Could you check a few things on this model? Use its own coordinates, in mm. A direction names the side the tool comes from. Give positions to 0.01 mm unless a question says otherwise; leave off trailing zeros. Order: outer loops, then holes, each group sorted by start corner. A loop starts at its lowest first (then second) coordinate and runs counter-clockwise, first axis right, second up. Notation, with made-up numbers: M 86.5,64.25 L 124.5,64.25 A27 cw 124.5,102.25 Z; hole C 52,46 d11. An arc over 180 degrees is marked long. Return JSON: item names as keys, results as strings. Group by question number.
```python
from build123d import *

# Parameters (mm, degrees)
CUT_EXTRUDE1_REACH = 152
SKETCH2_W          = 12
SKETCH2_H          = 6.6


with BuildPart() as part:
    # Sketch1 → Revolve1 (revolve)
    with BuildSketch(Plane.XY, mode=Mode.PRIVATE) as revolve1_sk:
        Polygon((-25, 21), (25, 21), (25, 30), (5, 30), (5, 90), (25, 90), (25, 100), (-25, 100), (-25, 90), (-5, 90), (-5, 30), (-25, 30), align=None)
    revolve(revolve1_sk.sketch.rotate(Axis((0, 0, 0), (1, 0, 0)), 90), axis=Axis((0, 0, 0), (1, 0, 0)))

    # Sketch2 → Cut-Extrude1 (cut, up to next)
    with BuildSketch(Plane(origin=(25, 0, 0), x_dir=(0, 0, -1), z_dir=(1, 0, 0)), mode=Mode.PRIVATE) as cut_extrude1_sk1:
        with Locations((0, 21)):
            Rectangle(SKETCH2_W, SKETCH2_H)
    cut_extrude1_tool1 = extrude(cut_extrude1_sk1.sketch, amount=-CUT_EXTRUDE1_REACH, mode=Mode.PRIVATE) & part.part
    add(cut_extrude1_tool1.solids().sort_by_distance((25, 21, 0))[0], mode=Mode.SUBTRACT)


solid = part.part
```
1. For pin 1 (25 mm diameter, centred on y = 0, z = 0, fed in from -X); pin 2 (3 mm diameter, centred on x = -11.5, z = -21.5, fed in from -Y); pin 3 (12 mm diameter, centred on x = -18.5, y = 41.5, fed in from -Z); pin 4 (1.5 mm diameter, centred on x = 19.5, z = -79.5, fed in from -Y), each with a flat end and sliding along its axis, tell me the tip position at first contact or that it passes through.
2. Imagine slicing it at A-A, the plane y = 0. Please give me the cut outline in (x, z), plus the area to 3 significant figures.
3. Imagine slicing it at D-D, the plane z = 77. Please give me the cut outline in (x, y), plus the area to 3 significant figures.
4. Imagine slicing it at B-B, the plane x = 15. Please give me the cut outline in (y, z).
5. Which directions (+Z, -Z, +X, -X, +Y, -Y) give clear straight access to the entire face, cutting with the end or side of a thin tool? Please do faces 4 (the cylindrical face through (14.86, -25.296, 16.128)), 5 (the flat face through (25, -20.4, -6.2)), 6 (the flat face through (0, 24.3, 0)), 7 (the flat face through (-5, 39, -1)).
6. I need wall thicknesses on L1, parallel to Y at x = -22, z = -0.5; L2, parallel to Z at x = 18, y = -3; L3, parallel to Z at x = -16, y = -9. Which ranges of each line are inside material? Lowest first, please. Write a range as from..to.
7. Imagine slicing it at C-C, the plane z = 0. Please give me the cut outline in (x, y).
8. If we mould it in two halves opening along Z, with no side actions, what happens to faces 1 (the cylindrical face through (0.35, -20.983, 0.838)), 2 (the cylindrical face through (-0.35, -30.04, 95.38)), 3 (the flat face through (-25, -38, -82))? For each: pulls with the +Z half, pulls with the -Z half, needs draft (parallel to the pull), parting line crosses it, or undercut.
Values:
{
 "1": {"pin 1": "passes through", "pin 2": "stops at y = -97.98", "pin 3": "stops at z = -93.49", "pin 4": "stops at y = -61.63"},
 "2": {"outline": "M -25,-100 L 25,-100 L 25,-90 L 5,-90 L 5,-30 L 25,-30 L 25,-21 L -25,-21 L -25,-30 L -5,-30 L -5,-90 L -25,-90 Z; M -25,21 L 25,21 L 25,30 L 5,30 L 5,90 L 25,90 L 25,100 L -25,100 L -25,90 L -5,90 L -5,30 L -25,30 Z", "area": "3,100 mm²"},
 "3": {"outline": "M -25,-63.8 L 25,-63.8 L 25,-46.59 L 5,-46.59 L 5,46.59 L 25,46.59 L 25,63.8 L -25,63.8 L -25,46.59 L -5,46.59 L -5,-46.59 L -25,-46.59 Z", "area": "2,650 mm²"},
 "4": {"outline": "C 0,0 d200; C 0,0 d60; hole C 0,0 d180; hole M 20.12,-6 L 24.3,-6 L 24.3,6 L 20.12,6 A21 ccw long Z"},
 "5": {"face 4": "+X", "face 5": "+Z, -Z, +X, +Y, -Y", "face 6": "+X, -X", "face 7": "-X"},
 "6": {"L1": "y = -100..-90, -30..-20.99, 24.3..30, 90..100", "L2": "z = -99.95..-89.95, -29.85..-20.78, 20.78..29.85, 89.95..99.95", "L3": "z = -99.59..-89.55, -28.62..-18.97, 18.97..28.62, 89.55..99.59"},
 "7": {"outline": "M -25,-100 L 25,-100 L 25,-90 L 5,-90 L 5,-30 L 25,-30 L 25,-21 L -25,-21 L -25,-30 L -5,-30 L -5,-90 L -25,-90 Z; M -25,24.3 L 25,24.3 L 25,30 L 5,30 L 5,90 L 25,90 L 25,100 L -25,100 L -25,90 L -5,90 L -5,30 L -25,30 Z"},
 "8": {"face 1": "undercut", "face 2": "parting line crosses it", "face 3": "needs draft"}
}
